Geometry check sheet. Reference: the model listing, model coordinates, mm. A direction names the side the tool comes from. Round coordinates to 2 decimals unless told otherwise and drop trailing zeros. Write each loop counter-clockwise with the first axis right and the second up, starting at its lowest first coordinate (ties: lowest second). Pieces come first, ordered by that corner, then holes. Notation, with made-up numbers: (-34, -35.75) -> (23, -35.75) arc R31 cw to (23, -6.75) -> close; hole circle Ø7 at (79.25, 79.25). An arc over 180 degrees is marked (long way). Use a Markdown table: item, result.
```python
from build123d import *

# Parameters (mm, degrees)
BOSS_EXTRUDE1_DEPTH   = 13
SKETCH2_W             = 2.5
SKETCH2_H             = 2.5
CUT_EXTRUDE1_DEPTH    = 118.749734607
M4_TAPPED_HOLE1_D     = 3.3
M4_TAPPED_HOLE1_DEPTH = 10.1
M3_TAPPED_HOLE1_D     = 2.5
M3_TAPPED_HOLE1_DEPTH = 7.5
CUT_EXTRUDE2_DEPTH    = 114.551750317
FILLET1_R             = 2
FILLET2_R             = 3
CHAMFER1_SIZE         = 2


with BuildPart() as part:
    # Sketch1 → Boss-Extrude1 (new, symmetric)
    with BuildSketch(Plane.XY):
        Polygon((0, 110), (8, 110), (8, 10), (33, 10), (33, 0), (0, 0), align=None)
    extrude(amount=BOSS_EXTRUDE1_DEPTH, both=True)

    # Sketch2 → Cut-Extrude1 (cut, through all)
    with BuildSketch(Plane.XY.offset(13)):
        with Locations((28.75, 1.25)):
            Rectangle(SKETCH2_W, SKETCH2_H)
    extrude(amount=-CUT_EXTRUDE1_DEPTH, mode=Mode.SUBTRACT)

    # M4 Tapped Hole1
    with Locations(Plane.XY.offset(13)):
        with Locations((21, 6), (4, 6)):
            m4_tapped_hole1 = Hole(M4_TAPPED_HOLE1_D / 2, depth=M4_TAPPED_HOLE1_DEPTH)

    # Mirror1: M4 Tapped Hole1 across plane
    add(m4_tapped_hole1.mirror(Plane.XY), mode=Mode.SUBTRACT)

    # M3 Tapped Hole1
    with Locations(Plane.XZ):
        with Locations((25, 8), (9, 8), (9, -8), (25, -8)):
            Hole(M3_TAPPED_HOLE1_D / 2, depth=M3_TAPPED_HOLE1_DEPTH)

    # Sketch7 → Cut-Extrude2 (cut, through all)
    with BuildSketch(Plane(origin=(8, 0, 0), x_dir=(0, 0, -1), z_dir=(1, 0, 0))):
        with BuildLine():
            Line((-3.75, 106), (-3.75, 98))
            ThreePointArc((-3.75, 98), (-6, 95.75), (-8.25, 98))
            Line((-8.25, 98), (-8.25, 106))
            ThreePointArc((-8.25, 106), (-6, 108.25), (-3.75, 106))
        make_face()
        with BuildLine():
            Line((3.75, 106), (3.75, 98))
            ThreePointArc((3.75, 98), (6, 95.75), (8.25, 98))
            Line((8.25, 98), (8.25, 106))
            ThreePointArc((8.25, 106), (6, 108.25), (3.75, 106))
        make_face()
    extrude(amount=-CUT_EXTRUDE2_DEPTH, mode=Mode.SUBTRACT)

    # Fillet1
    fillet1_edges = [part.edges().sort_by_distance(p)[0] for p in [
        (33, 0, 0),
    ]]
    fillet(fillet1_edges, radius=FILLET1_R)

    # Fillet2
    fillet2_edges = [part.edges().sort_by_distance(p)[0] for p in [
        (8, 10, 0),
    ]]
    fillet(fillet2_edges, radius=FILLET2_R)

    # Chamfer1
    chamfer1_edges = [part.edges().sort_by_distance(p)[0] for p in [
        (4, 110, 13),
        (4, 110, -13),
    ]]
    chamfer(chamfer1_edges, length=CHAMFER1_SIZE)


solid = part.part
```
(1) Section check D-D on x = 21. Record the cut outline in (y, z), plus the area to 3 significant figures.
A:
| item | result |
|---|---|
| outline | (0, -13) -> (4.35, -13) -> (4.35, -2.9) -> (7.65, -2.9) -> (7.65, -13) -> (10, -13) -> (10, 13) -> (7.65, 13) -> (7.65, 2.9) -> (4.35, 2.9) -> (4.35, 13) -> (0, 13) -> close |
| area | 193 mm2 |
(2) Thickness scan on line 1 (Y direction, x = 21, z = 8.25); line 2 (X direction, y = 6, z = -7.25); line 3 (X direction, y = 6, z = -7). Record the ranges inside material, lowest first.
A:
| item | result |
|---|---|
| line 1 | y = 0 to 4.35, 7.65 to 10 |
| line 2 | x = 0 to 2.35, 5.65 to 8, 10 to 19.35, 22.65 to 24, 26 to 33 |
| line 3 | x = 0 to 2.35, 5.65 to 8.25, 9.75 to 19.35, 22.65 to 24.25, 25.75 to 33 |
(3) Gauge pin test, flat ends, axial feed: pin 1 Ø1.2 at (x, z) = (9, 8) entering from -Y; pin 2 Ø6 at (y, z) = (17, -4) entering from +X; pin 3 Ø8 at (x, y) = (12.5, 31.5) entering from -Z; pin 4 Ø3 at (x, y) = (21, 6) entering from +Z. Record the tip position at first contact, or that the pin passes through.
A:
| item | result |
|---|---|
| pin 1 | stops at y = 7.5 |
| pin 2 | stops at x = 8 |
| pin 3 | passes through |
| pin 4 | stops at z = 2.9 |
(4) Access from +Z, -Z, +X, -X, +Y, -Y to the whole of each face (thin tool, end or side, straight path). Record for faces 1 (the face through (27.5, 1, 0)), 2 (the face through (4, 102, 8.25)), 3 (the face through (4, 6, 2.9)).
A:
| item | result |
|---|---|
| face 1 | +Z, -Z, -Y |
| face 2 | +X, -X |
| face 3 | +Z |
(5) Section check A-A on y = 6. Record the cut outline in (x, z).
A:
| item | result |
|---|---|
| outline | (0, -13) -> (2.35, -13) -> (2.35, -2.9) -> (5.65, -2.9) -> (5.65, -13) -> (19.35, -13) -> (19.35, -2.9) -> (22.65, -2.9) -> (22.65, -13) -> (33, -13) -> (33, 13) -> (22.65, 13) -> (22.65, 2.9) -> (19.35, 2.9) -> (19.35, 13) -> (5.65, 13) -> (5.65, 2.9) -> (2.35, 2.9) -> (2.35, 13) -> (0, 13) -> close; hole circle Ø2.5 at (9, -8); hole circle Ø2.5 at (9, 8); hole circle Ø2.5 at (25, -8); hole circle Ø2.5 at (25, 8) |
(6) Section check C-C on x = 4. Record the cut outline in (y, z), plus the area to 3 significant figures.
A:
| item | result |
|---|---|
| outline | (0, -13) -> (4.35, -13) -> (4.35, -2.9) -> (7.65, -2.9) -> (7.65, -13) -> (108, -13) -> (110, -11) -> (110, 11) -> (108, 13) -> (7.65, 13) -> (7.65, 2.9) -> (4.35, 2.9) -> (4.35, 13) -> (0, 13) -> close; hole (98, -8.25) -> (106, -8.25) arc R2.25 ccw to (106, -3.75) -> (98, -3.75) arc R2.25 ccw to start; hole (98, 3.75) -> (106, 3.75) arc R2.25 ccw to (106, 8.25) -> (98, 8.25) arc R2.25 ccw to start |
| area | 2,690 mm2 |
(7) Section check B-B on z = 5.5. Record the cut outline in (x, y), plus the area to 3 significant figures.
A:
| item | result |
|---|---|
| outline | (0, 0) -> (27.5, 0) -> (27.5, 2.5) -> (30, 2.5) -> (30, 0) -> (31, 0) arc R2 ccw to (33, 2) -> (33, 10) -> (11, 10) arc R3 cw to (8, 13) -> (8, 95.81) -> (0, 95.81) -> close; (0, 108.19) -> (8, 108.19) -> (8, 110) -> (0, 110) -> close; hole circle Ø3.3 at (4, 6); hole circle Ø3.3 at (21, 6) |
| area | 1,010 mm2 |
(8) Release check for a two-part mould opening along Z. For faces 4 (the face through (4, 110, 0)), 5 (the face through (4, 109, 12)), 6 (the face through (4.06, 95.75, -5.95)) record: +Z half, -Z half, draft (parallel to the pull), parting line (faces both ways), or undercut.
A:
| item | result |
|---|---|
| face 4 | draft |
| face 5 | +Z half |
| face 6 | undercut |
